from build123d import *

# Parameters (mm, degrees)
SKETCH_1_W                   = 90
SKETCH_1_H                   = 30
EXTRUDE_1_DEPTH              = 11.5
HOLE_WIZARD_M4_1_D           = 4.5
HOLE_WIZARD_M4_1_CBORE_D     = 8
HOLE_WIZARD_M4_1_CBORE_DEPTH = 4.4
FILLET_1_R                   = 3


with BuildPart() as part:
    # 草图1 → 凸台-拉伸1 (new, symmetric)
    with BuildSketch(Plane(origin=(0, 0, 0), x_dir=(1, 0, 0), z_dir=(0, 1, 0))):
        Rectangle(SKETCH_1_W, SKETCH_1_H)
    extrude(amount=EXTRUDE_1_DEPTH, both=True)

    # M4 六角凹头螺钉的柱形沉头孔1 (through all)
    with Locations(Plane(origin=(0, 11.5, 0), x_dir=(1, 0, 0), z_dir=(0, 1, 0))):
        with Locations((-40, 0), (40, 0)):
            CounterBoreHole(HOLE_WIZARD_M4_1_D / 2, HOLE_WIZARD_M4_1_CBORE_D / 2, HOLE_WIZARD_M4_1_CBORE_DEPTH)

    # 圆角1
    fillet_1_edges = [part.edges().sort_by_distance(p)[0] for p in [
        (45, 0, 15),
        (-45, 0, 15),
        (-45, 0, -15),
        (45, 0, -15),
    ]]
    fillet(fillet_1_edges, radius=FILLET_1_R)


solid = part.part
Could you check a few things on this model? Use its own coordinates, in mm. A direction names the side the tool comes from. Give positions to 0.01 mm unless a question says otherwise; leave off trailing zeros. Write each loop counter-clockwise with the first axis right and the second up, starting at its lowest first coordinate (ties: lowest second). Pieces come first, ordered by that corner, then holes. Notation, with made-up numbers: (17, -11.5) -> (47, -11.5) arc R18 ccw to (47, 3.5) -> close; hole circle Ø10 at (60, -15). An arc over 180 degrees is marked (long way). Write each question's results on one line, items separated by ' | '. Start each with the question number.
Q1. Suppose I cut it at B-B, the plane y = 8.25. List the corners of the cut face in (x, z) for me, and give its area (3 significant figures).
Q2. Which directions (+Z, -Z, +X, -X, +Y, -Y) give clear straight access to the entire face, cutting with the end or side of a thin tool? Please do faces 4 (the face through (36.8, 9.3, 2.4)), 5 (the face through (-1, -11.5, 0)).
Q3. I need wall thicknesses on probe 1 along Z at (x, y) = (40, 2); probe 2 along X at (y, z) = (-2, 0.25); probe 3 along Z at (x, y) = (-40, 8). Which ranges of each line are inside material? Lowest first, please.
Q4. I'm going to push a flat-ended pin straight in: pin 1 Ø4 at (x, z) = (41.5, 0.5) entering from +Y. Where does the tip first touch, or does it pass through?
Q5. We'd pull the mould along X, two halves only. Please class faces 1 (the face through (-1, 11.5, 0)), 2 (the face through (-44.14, -0.16, -14.1)), 3 (the face through (-37.752, -2.33, -0.099)): +X half, -X half, draft (parallel to the pull), parting line (faces both ways), or undercut.
Q6. Suppose I cut it at C-C, the plane x = -40. List the corners of the cut face in (y, z) for me, and give its area (3 significant figures).
Q7. Suppose I cut it at A-A, the plane z = 0. List the corners of the cut face in (x, y) for me, and give its area (3 significant figures).
Outcome:
1) outline: (-45, -12) arc R3 ccw to (-42, -15) -> (42, -15) arc R3 ccw to (45, -12) -> (45, 12) arc R3 ccw to (42, 15) -> (-42, 15) arc R3 ccw to (-45, 12) -> close; hole circle Ø8 at (-40, 0); hole circle Ø8 at (40, 0) | area: 2,590 mm2
2) face 4: +Y | face 5: +Z, -Z, +X, -X, -Y
3) probe 1: -15 to -2.25, 2.25 to 15 | probe 2: -45 to -42.24, -37.76 to 37.76, 42.24 to 45 | probe 3: -15 to -4, 4 to 15
4) pin 1: y = 7.1
5) face 1: draft | face 2: -X half | face 3: undercut
6) outline: (-11.5, -15) -> (11.5, -15) -> (11.5, -4) -> (7.1, -4) -> (7.1, -2.25) -> (-11.5, -2.25) -> close; (-11.5, 2.25) -> (7.1, 2.25) -> (7.1, 4) -> (11.5, 4) -> (11.5, 15) -> (-11.5, 15) -> close | area: 571 mm2
7) outline: (-45, -11.5) -> (-42.25, -11.5) -> (-42.25, 7.1) -> (-44, 7.1) -> (-44, 11.5) -> (-45, 11.5) -> close; (-37.75, -11.5) -> (37.75, -11.5) -> (37.75, 7.1) -> (36, 7.1) -> (36, 11.5) -> (-36, 11.5) -> (-36, 7.1) -> (-37.75, 7.1) -> close; (42.25, -11.5) -> (45, -11.5) -> (45, 11.5) -> (44, 11.5) -> (44, 7.1) -> (42.25, 7.1) -> close | area: 1,830 mm2
